The drawing under review shows one solid part. Ordinate dimensions are in mm from its lowest x, y, z. A direction names the side the tool comes from. Coordinates: 2 decimals unless noted, no trailing zeros. Write each loop counter-clockwise with the first axis right and the second up, starting at its lowest first coordinate (ties: lowest second). Pieces come first, ordered by that corner, then holes.
Q1. For probe 1 along Y at (x, z) = (66, 5); probe 2 along X at (y, z) = (49.5, 52); probe 3 along Z at (x, y) = (23, 12), list the stretches that pass through material, from the lowest coordinate up.
Q2. Machinability: for the marked faces 1, 2, 3 and 4, which of the approach directions +Z, -Z, +X, -X, +Y, -Y give a long, thin tool a straight path to every point of the face, cutting with its end or side? Answer none if there is none.
Q3. Mouldability with a two-part tool opening along Z and no side actions: class the marked faces 5, 6 and 7 as pulls with the +Z half, pulls with the -Z half, needs draft (parallel to the pull), parting line crosses it, or undercut.
Q4. Take a section at B-B (z = 59). Give the boundary of the cut face in (x, y), and give its area (3 significant figures).
Q5. Take a section at A-A (y = 19). Give the boundary of the cut face in (x, z), and give its area (3 significant figures).
Q6. Take a section at D-D (x = 121). Give the boundary of the cut face in (y, z), and give its area (3 significant figures).
Q7. Take a section at C-C (y = 11). Give the boundary of the cut face in (x, z), and give its area (3 significant figures).
Q8. Insertion check: pin 1 (4 mm diameter, centred on y = 5.5, z = 26.5, fed in from +X); pin 2 (10 mm diameter, centred on x = 115, z = 34.5, fed in from -Y); pin 3 (8 mm diameter, centred on x = 48.5, z = 65, fed in from -Y). Each pin has a flat end and moves straight along its axis. Give the tip position at first contact, or say it passes through.
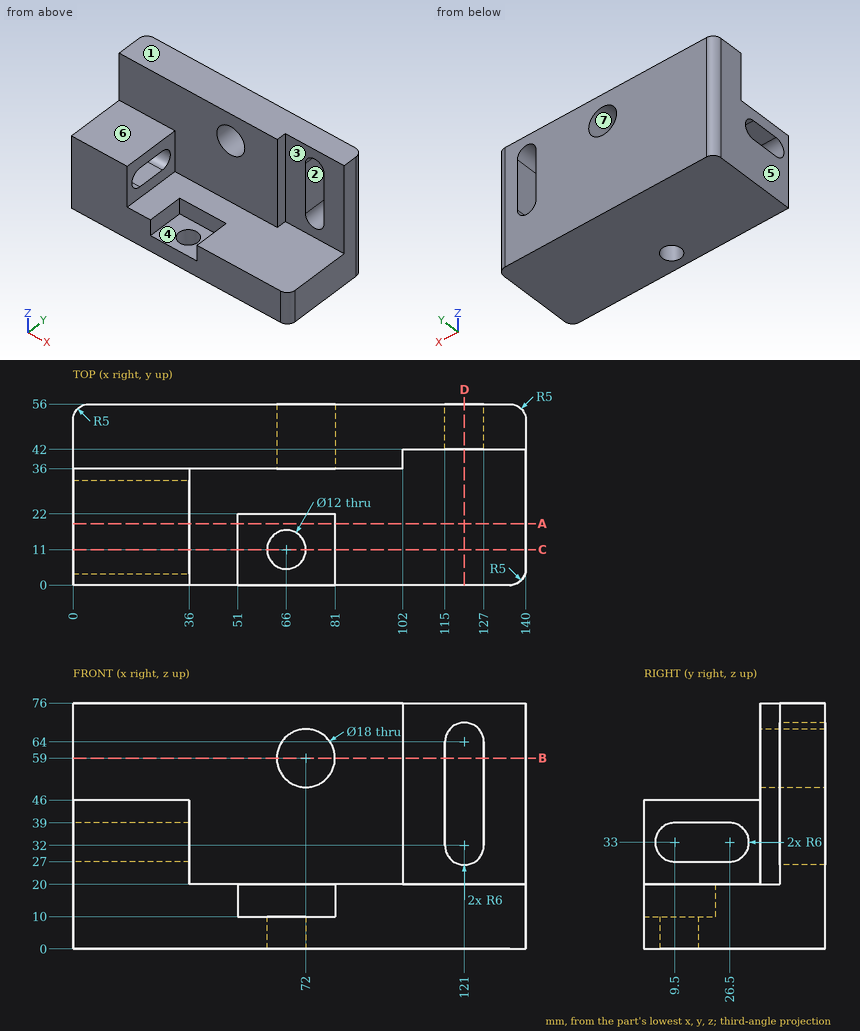
Response:
1. probe 1: y = 0 to 5, 17 to 56
1. probe 2: x = 0 to 66.34, 77.66 to 115, 127 to 140
1. probe 3: z = 0 to 27, 39 to 46
2. face 1: +Z, +X, -X, +Y, -Y
2. face 2: +Y, -Y
2. face 3: +Z, +X, -Y
2. face 4: +Z, -Y
3. face 5: needs draft
3. face 6: pulls with the +Z half
3. face 7: undercut
4. outline: (0, 36) - (63, 36) - (63, 56) - (5, 56) arc R5 ccw to (0, 51) - close; (81, 36) - (102, 36) - (102, 42) - (115, 42) - (115, 56) - (81, 56) - close; (127, 42) - (140, 42) - (140, 51) arc R5 ccw to (135, 56) - (127, 56) - close
4. area: 2,030 mm2
5. outline: (0, 0) - (140, 0) - (140, 20) - (81, 20) - (81, 10) - (51, 10) - (51, 20) - (36, 20) - (36, 27) - (0, 27) - close; (0, 39) - (36, 39) - (36, 46) - (0, 46) - close
5. area: 3,000 mm2
6. outline: (0, 0) - (56, 0) - (56, 26) - (42, 26) - (42, 20) - (0, 20) - close; (42, 70) - (56, 70) - (56, 76) - (42, 76) - close
6. area: 1,290 mm2
7. outline: (0, 0) - (60, 0) - (60, 10) - (51, 10) - (51, 20) - (36, 20) - (36, 27) - (0, 27) - close; (0, 39) - (36, 39) - (36, 46) - (0, 46) - close; (72, 0) - (140, 0) - (140, 20) - (81, 20) - (81, 10) - (72, 10) - close
7. area: 2,880 mm2
8. pin 1: stops at x = 36
8. pin 2: stops at y = 42
8. pin 3: stops at y = 36
